Answer from the drawing. Dimensions are ordinates in mm from the lowest x, y and z of the part. A direction names the side the tool comes from. Round coordinates to 2 decimals unless told otherwise and drop trailing zeros. Loops run counter-clockwise (first coordinate to the right, second up) from the corner with the lowest first, then second, coordinate; pieces in that order, holes last. Notation, with made-up numbers: (78, 38.25) -> (121, 38.25) arc R23 cw to (121, 50.25) -> close; hole circle Ø10 at (55, -15.5). An arc over 180 degrees is marked (long way). One line per question, with ' | ' between items.
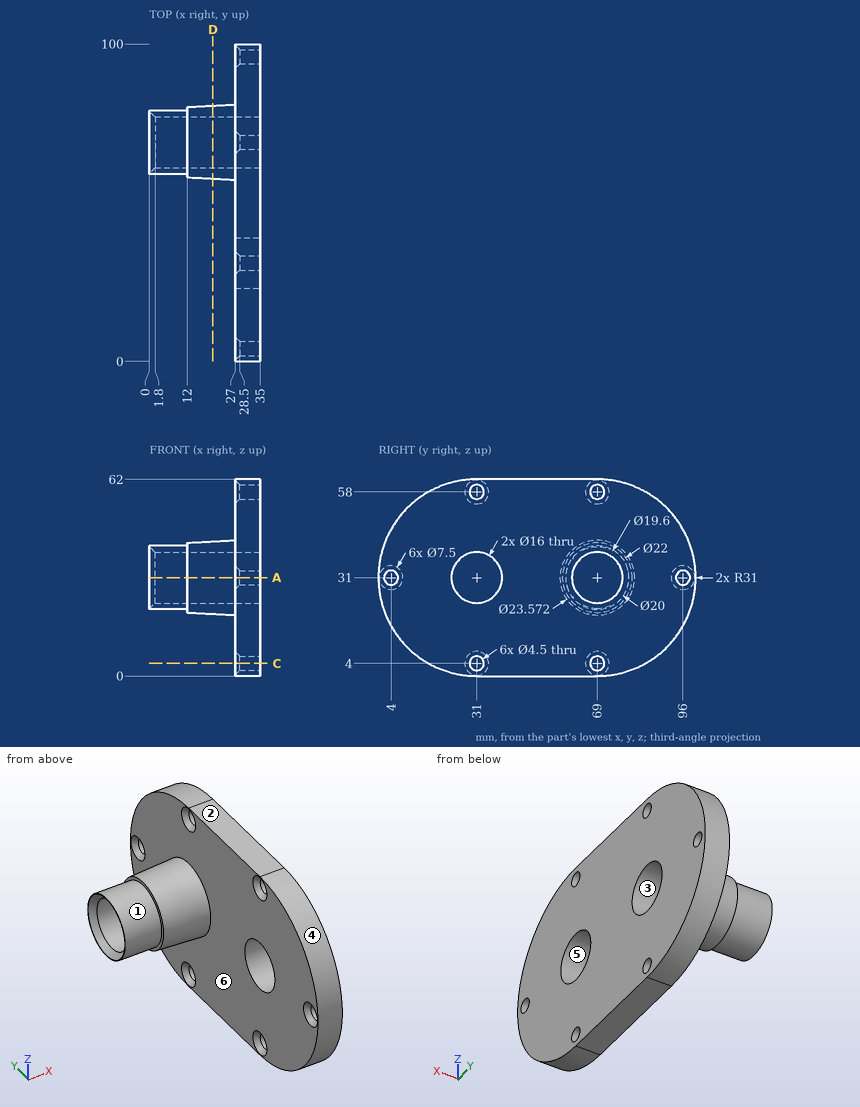
Q1. A cutting plane is placed at A-A on z = 31. Give the number of separate pieces and of enclosed holes in the cut face, plus the area to 3 significant figures.
Numbers:
separate pieces: 5 | enclosed holes: 0 | area: 614 mm^2
Q2. A cutting plane is placed at C-C on z = 4. Give the vertices of the cut face in (x, y), plus the area to 3 significant figures.
Numbers:
outline: (27, 15.77) -> (35, 15.77) -> (35, 28.75) -> (28.5, 28.75) -> (27, 27.25) -> close; (27, 34.75) -> (28.5, 33.25) -> (35, 33.25) -> (35, 66.75) -> (28.5, 66.75) -> (27, 65.25) -> close; (27, 72.75) -> (28.5, 71.25) -> (35, 71.25) -> (35, 84.23) -> (27, 84.23) -> close | area: 471 mm^2
Q3. For the marked faces 1 and 2, determine the directions among +Z, -Z, +X, -X, +Y, -Y from which every point of the face is accessible in a straight line to the end or side of a thin tool.
Numbers:
face 1: -X | face 2: +Z, +X, -X, +Y, -Y
Q4. For a pull along Z with two mould halves and no side action, classify the marked faces 3, 4, 5 and 6 as pulls with the +Z half, pulls with the -Z half, needs draft (parallel to the pull), parting line crosses it, or undercut.
Numbers:
face 3: undercut | face 4: parting line crosses it | face 5: undercut | face 6: needs draft
Q5. Given pin 1 Ø7 at (y, z) = (31, 4) entering from -X; pin 2 Ø5 at (y, z) = (25.5, 9) entering from -X; pin 3 Ø4 at (y, z) = (69, 4) entering from -X; pin 4 Ø6 at (y, z) = (4, 31) entering from -X, each flat-ended and moving along its own axis, determine where each tip first touches the part or whether it passes through.
Numbers:
pin 1: x = 27.25 | pin 2: x = 27 | pin 3: through | pin 4: x = 27.75
Q6. Find the intervals of material crossed by line 1 (Y direction, x = 31, z = 31); line 2 (Y direction, x = 31, z = 58); line 3 (X direction, y = 31, z = 48), in increasing order. Write a range as from..to.
Numbers:
line 1: 0..1.75, 6.25..23, 39..61, 77..93.75, 98.25..100 | line 2: 15.77..28.75, 33.25..66.75, 71.25..84.23 | line 3: 27..35
Q7. A cutting plane is placed at D-D on x = 20. Give the vertices of the cut face in (y, z), plus the area to 3 significant figures.
Numbers:
outline: circle Ø22.84 at (69, 31); hole circle Ø16 at (69, 31) | area: 209 mm^2
